Could you check a few things on this drawing? It's one solid part, dimensions in mm from its lowest x, y, z. Give positions to 0.01 mm unless a question says otherwise; leave off trailing zeros. Write each loop counter-clockwise with the first axis right and the second up, starting at its lowest first coordinate (ties: lowest second). Pieces come first, ordered by that corner, then holes. Notation, with made-up numbers: M 17,-32 L 55,-32 A18 cw 55,-14 Z; hole C 27,62 d4. An arc over 180 degrees is marked long. Use CSV: the item, a comma, the result in double quotes. Start each with the question number.
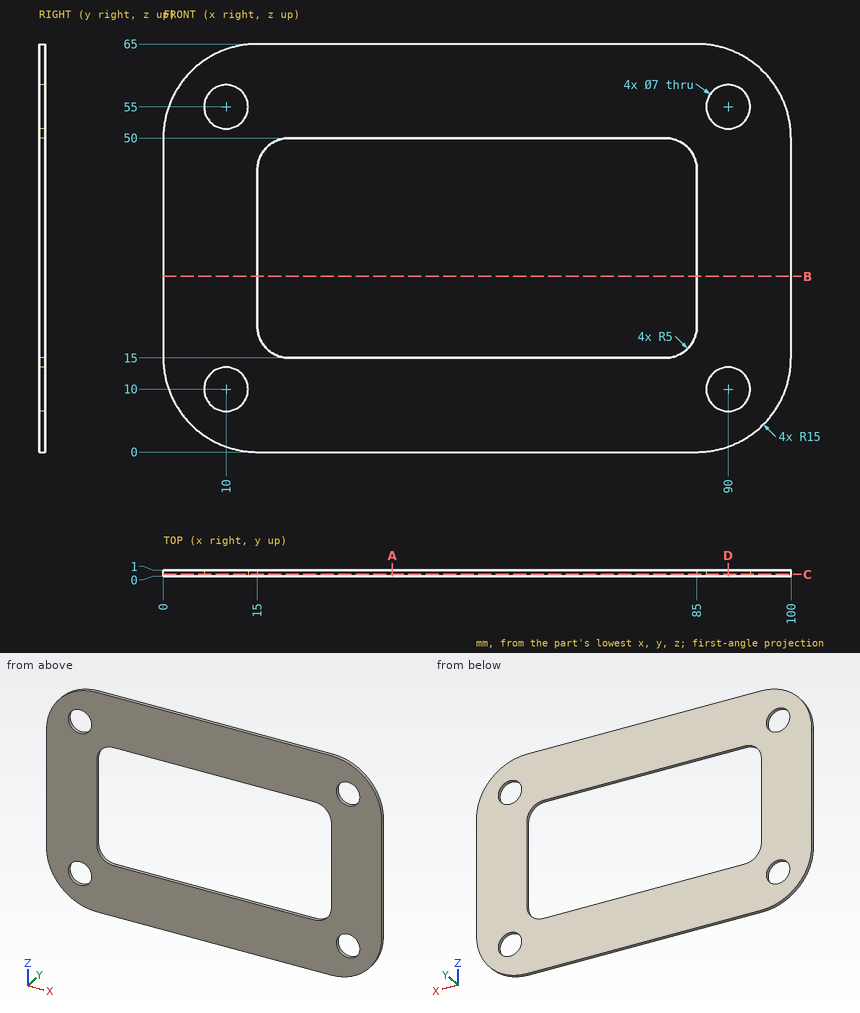
(1) I want a section at D-D (x = 90). Write out the boundary of the cut face in (y, z), and give its area (3 significant figures).
(2) Will these pins go through, and if not, where does the flat tip stop? pin 1 Ø6.5 at (x, z) = (10, 10) entering from +Y; pin 2 Ø4 at (x, z) = (57.5, 15.5) entering from +Y.
(3) Please list where these lines run through material, in increasing order: L1, parallel to X at y = 0.7, z = 33.5; L2, parallel to X at y = 0.75, z = 55; L3, parallel to Z at x = 21.5, y = 0.4. Write a range as [from, to].
(4) I want a section at C-C (y = 0.3). Write out the boundary of the cut face in (x, z).
(5) I want a section at B-B (z = 28). Write out the boundary of the cut face in (x, y), and give its area (3 significant figures).
(6) I want a section at A-A (x = 36.5). Write out the boundary of the cut face in (y, z), and give its area (3 significant figures).
Geometry results:
1,outline,"M 0,0.86 L 1,0.86 L 1,6.5 L 0,6.5 Z; M 0,13.5 L 1,13.5 L 1,51.5 L 0,51.5 Z; M 0,58.5 L 1,58.5 L 1,64.14 L 0,64.14 Z"
1,area,"49.3 mm2"
2,pin 1,"passes through"
2,pin 2,"stops at y = 1"
3,L1,"x = [0, 15], [85, 100]"
3,L2,"x = [0.86, 6.5], [13.5, 86.5], [93.5, 99.14]"
3,L3,"z = [0, 15], [50, 65]"
4,outline,"M 0,15 A15 ccw 15,0 L 85,0 A15 ccw 100,15 L 100,50 A15 ccw 85,65 L 15,65 A15 ccw 0,50 Z; hole C 10,10 d7; hole C 10,55 d7; hole M 15,20 A5 ccw 20,15 L 80,15 A5 ccw 85,20 L 85,45 A5 ccw 80,50 L 20,50 A5 ccw 15,45 Z; hole C 90,10 d7; hole C 90,55 d7"
5,outline,"M 0,0 L 15,0 L 15,1 L 0,1 Z; M 85,0 L 100,0 L 100,1 L 85,1 Z"
5,area,"30.0 mm2"
6,outline,"M 0,0 L 1,0 L 1,15 L 0,15 Z; M 0,50 L 1,50 L 1,65 L 0,65 Z"
6,area,"30.0 mm2"
